Input: dimensioned drawing with shaded views. Units: mm. Origin: part minimum x, y, z. Coordinates: 2 decimals unless noted, no trailing zeros. Loops run counter-clockwise (first coordinate to the right, second up) from the corner with the lowest first, then second, coordinate; pieces in that order, holes last. Notation, with made-up numbers: (33, 48.25) - (71, 48.25) arc R14 cw to (71, 56.25) - close; hole circle Ø2 at (-21.5, 80.5). An arc over 180 degrees is marked (long way). Use one line per item in the form item = value. Start each with the question number.
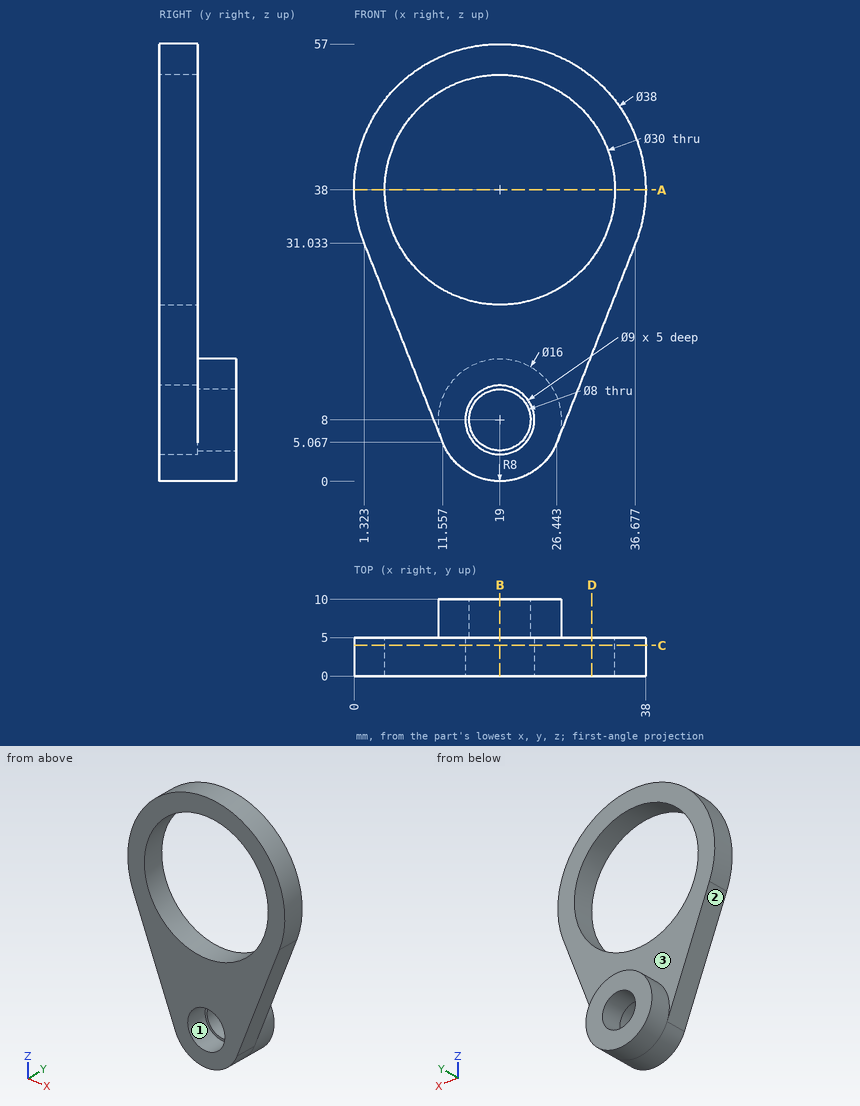
(1) Cut plane D-D, the plane x = 31. Output: boundary loops of the cut face in (y, z).
(2) Material intervals for line 1 (Z direction, x = 18.5, y = 2.25) (1 decimal); line 2 (X direction, y = 2.45, z = 8); line 3 (Z direction, x = 18, y = 5.25), sorted ascending.
(3) Cut plane C-C, the plane y = 4. Output: boundary loops of the cut face in (x, z).
(4) Mould query, pull axis Z, two halves, no side actions, for the marked faces 1, 2 and 3. Classes: +Z half, -Z half, draft (parallel to the pull), parting line (faces both ways), or undercut.
(5) Cut plane B-B, the plane x = 19. Output: boundary loops of the cut face in (y, z), plus the area to 3 significant figures.
(6) Cut plane A-A, the plane z = 38. Output: boundary loops of the cut face in (x, y), plus the area to 3 significant figures.
(7) Contact query for flat-ended pins moving along their axis: pin 1 (4 mm diameter, centred on x = 7.5, y = 2, fed in from +Z) (1 decimal); pin 2 (1.5 mm diameter, centred on x = 17.5, z = 6, fed in from +Y); pin 3 (4 mm diameter, centred on y = 5.5, z = 31.5, fed in from -X); pin 4 (3 mm diameter, centred on x = 9, z = 26.5, fed in from +Y). Output: stop coordinate, or through.
Recorded:
q1.outline = (0, 16.63) - (5, 16.63) - (5, 29) - (0, 29) - close; (0, 47) - (5, 47) - (5, 52.73) - (0, 52.73) - close
q2.line_1 = 0 to 3.5, 12.5 to 23, 53 to 57
q2.line_2 = 10.4 to 14.5, 23.5 to 27.6
q2.line_3 = 0.06 to 4.13, 11.87 to 15.94
q3.outline = (1.32, 31.03) - (11.56, 5.07) arc R8 ccw to (26.44, 5.07) - (36.68, 31.03) arc R19 ccw (long way) to start; hole circle Ø30 at (19, 38); hole circle Ø9 at (19, 8)
q4.face_1 = undercut
q4.face_2 = -Z half
q4.face_3 = draft
q5.outline = (0, 0) - (10, 0) - (10, 4) - (5, 4) - (5, 3.5) - (0, 3.5) - close; (0, 12.5) - (5, 12.5) - (5, 12) - (10, 12) - (10, 16) - (5, 16) - (5, 23) - (0, 23) - close; (0, 53) - (5, 53) - (5, 57) - (0, 57) - close
q5.area = 130 mm²
q6.outline = (0, 0) - (4, 0) - (4, 5) - (0, 5) - close; (34, 0) - (38, 0) - (38, 5) - (34, 5) - close
q6.area = 40.0 mm²
q7.pin_1 = 54.5
q7.pin_2 = through
q7.pin_3 = 0.56
q7.pin_4 = 5
